Verification items for the finished model (mm, model axes). A direction names the side the tool comes from. Round coordinates to 2 decimals unless told otherwise and drop trailing zeros. Order: outer loops, then holes, each group sorted by start corner. A loop starts at its lowest first (then second) coordinate and runs counter-clockwise, first axis right, second up. Notation, with made-up numbers: (48.25, -22) -> (74.25, -22) arc R18 ccw to (74.25, 0) -> close; hole circle Ø4 at (51, 29.25). An arc over 180 degrees is marked (long way). Put each result on its own line as item: value.
from build123d import *

# Parameters (mm, degrees)
SQUARE_FLANGE_SKETCH_R           = 1
SQUARE_FLANGE_SKETCH_R_2         = 0.265
SQUARE_OUTLET_FLANGE_DEPTH       = 0.65
ROUND_FLANGE_HOLES_SKETCH_R      = 0.375
ROUND_FLANGE_HOLES_4X_0_75_DEPTH = 0.65
ROUND_FLANGE_HOLE_CHAMFERS_SIZE  = 0.0325
SQUARE_FLANGE_CHAMFERS_SIZE      = 0.0325
HOUSING_EDGE_CHAMFERS_SIZE       = 0.125


with BuildPart() as part:
    # Housing Profile Sketch → Housing Body Revolve (revolve)
    with BuildSketch(Plane.XY, mode=Mode.PRIVATE) as housing_body_revolve_sk:
        Polygon((0, 1), (0, 1.8125), (0.063, 1.8755), (0.063, 3), (0.65, 3), (0.65, 1.504103507), (1.375, 1.35), (2.125, 1.35), (2.125, 1.812), (2.188, 1.875), (2.188, 1), align=None)
    revolve(housing_body_revolve_sk.sketch.rotate(Axis((0, 0, 0), (1, 0, 0)), 90), axis=Axis((0, 0, 0), (1, 0, 0)))

    # Square Flange Sketch → Square Outlet Flange (add)
    with BuildSketch(Plane(origin=(2.188, 0, 0), x_dir=(0, 0, -1), z_dir=(1, 0, 0))):
        with BuildLine():
            Line((-1.594555277, 2.361757009), (-1.047699115, 2.375349419))
            ThreePointArc((-1.047699115, 2.375349419), (-0.801459389, 2.393837984), (-0.558303573, 2.436862146))
            ThreePointArc((-0.558303573, 2.436862146), (0.0283118, 2.499839683), (0.613350393, 2.423592642))
            ThreePointArc((0.613350393, 2.423592642), (0.974691231, 2.360294751), (1.341424141, 2.351306033))
            Line((1.341424141, 2.351306033), (1.535705916, 2.361018432))
            ThreePointArc((1.535705916, 2.361018432), (2.110295851, 2.15191191), (2.361757009, 1.594555277))
            Line((2.361757009, 1.594555277), (2.375349419, 1.047699115))
            ThreePointArc((2.375349419, 1.047699115), (2.393837984, 0.801459389), (2.436862146, 0.558303573))
            ThreePointArc((2.436862146, 0.558303573), (2.499839683, -0.0283118), (2.423592642, -0.613350393))
            ThreePointArc((2.423592642, -0.613350393), (2.360294751, -0.974691231), (2.351306033, -1.341424141))
            Line((2.351306033, -1.341424141), (2.361018432, -1.535705916))
            ThreePointArc((2.361018432, -1.535705916), (2.15191191, -2.110295851), (1.594555277, -2.361757009))
            Line((1.594555277, -2.361757009), (1.047699115, -2.375349419))
            ThreePointArc((1.047699115, -2.375349419), (0.801459389, -2.393837984), (0.558303573, -2.436862146))
            ThreePointArc((0.558303573, -2.436862146), (-0.0283118, -2.499839683), (-0.613350393, -2.423592642))
            ThreePointArc((-0.613350393, -2.423592642), (-0.974691231, -2.360294751), (-1.341424141, -2.351306033))
            Line((-1.341424141, -2.351306033), (-1.535705916, -2.361018432))
            ThreePointArc((-1.535705916, -2.361018432), (-2.110295851, -2.15191191), (-2.361757009, -1.594555277))
            Line((-2.361757009, -1.594555277), (-2.375349419, -1.047699115))
            ThreePointArc((-2.375349419, -1.047699115), (-2.393837984, -0.801459389), (-2.436862146, -0.558303573))
            ThreePointArc((-2.436862146, -0.558303573), (-2.499839683, 0.0283118), (-2.423592642, 0.613350393))
            ThreePointArc((-2.423592642, 0.613350393), (-2.360294751, 0.974691231), (-2.351306033, 1.341424141))
            Line((-2.351306033, 1.341424141), (-2.361018432, 1.535705916))
            ThreePointArc((-2.361018432, 1.535705916), (-2.15191191, 2.110295851), (-1.594555277, 2.361757009))
        make_face()
        with Locations(Location((0, 0, 0), (0, 0, 180))):
            Circle(SQUARE_FLANGE_SKETCH_R, mode=Mode.SUBTRACT)
        with Locations((-1.679378605, 1.679378605)):
            Circle(SQUARE_FLANGE_SKETCH_R_2, mode=Mode.SUBTRACT)
        with Locations((1.679378605, 1.679378605)):
            Circle(SQUARE_FLANGE_SKETCH_R_2, mode=Mode.SUBTRACT)
        with Locations((1.679378605, -1.679378605)):
            Circle(SQUARE_FLANGE_SKETCH_R_2, mode=Mode.SUBTRACT)
        with Locations((-1.679378605, -1.679378605)):
            Circle(SQUARE_FLANGE_SKETCH_R_2, mode=Mode.SUBTRACT)
    extrude(amount=SQUARE_OUTLET_FLANGE_DEPTH)

    # Round Flange Holes Sketch → Round Flange Holes 4xØ0.75 (cut)
    with BuildSketch(Plane.ZY.offset(-0.063)):
        with Locations((-1.575, 1.777638883)):
            Circle(ROUND_FLANGE_HOLES_SKETCH_R)
        with Locations((1.777638883, 1.575)):
            Circle(ROUND_FLANGE_HOLES_SKETCH_R)
        with Locations((1.575, -1.777638883)):
            Circle(ROUND_FLANGE_HOLES_SKETCH_R)
        with Locations((-1.777638883, -1.575)):
            Circle(ROUND_FLANGE_HOLES_SKETCH_R)
    extrude(amount=-ROUND_FLANGE_HOLES_4X_0_75_DEPTH, mode=Mode.SUBTRACT)

    # Round Flange Hole Chamfers
    round_flange_hole_chamfers_edges = [part.edges().sort_by_distance(p)[0] for p in [
        (0.65, -1.777638883, 1.2),
        (0.063, -1.777638883, 1.2),
        (0.65, 1.575, 1.402638883),
        (0.063, 1.575, 1.402638883),
        (0.65, 1.777638883, -1.95),
        (0.063, 1.777638883, -1.95),
        (0.65, -1.575, -2.152638883),
        (0.063, -1.575, -2.152638883),
    ]]
    chamfer(round_flange_hole_chamfers_edges, length=ROUND_FLANGE_HOLE_CHAMFERS_SIZE)

    # Square Flange Chamfers
    square_flange_chamfers_edges = [part.edges().sort_by_distance(p)[0] for p in [
        (2.188, 1.679378605, 1.944378605),
        (2.188, 1.679378605, -1.414378605),
        (2.188, -1.679378605, -1.414378605),
        (2.188, -1.679378605, 1.944378605),
        (2.838, 1.679378605, 1.944378605),
        (2.838, 1.679378605, -1.414378605),
        (2.838, -1.679378605, -1.414378605),
        (2.838, -1.679378605, 1.944378605),
    ]]
    chamfer(square_flange_chamfers_edges, length=SQUARE_FLANGE_CHAMFERS_SIZE)

    # Housing Edge Chamfers
    housing_edge_chamfers_edges = [part.edges().sort_by_distance(p)[0] for p in [
        (0, 0, -1),
        (2.838, 0, -1),
    ]]
    chamfer(housing_edge_chamfers_edges, length=HOUSING_EDGE_CHAMFERS_SIZE)


solid = part.part
Item 1: Gauge pin test, flat end, axial feed: pin 1 Ø1.5 at (x, z) = (1, -1) entering from -Y. Record the tip position at first contact, or that the pin passes through.
Check sheet entries:
pin 1: stops at y = -2.98
Item 2: Release check for a two-part mould opening along Z. For faces 1 (the cylindrical face through (0.36, -0.9, 2.86)), 2 (the flat face through (0, 1, 1)), 3 (the cylindrical face through (1, 1, 0)) record: +Z half, -Z half, draft (parallel to the pull), parting line (faces both ways), or undercut.
Check sheet entries:
face 1: parting line
face 2: draft
face 3: undercut
Item 3: Material ranges on L1, parallel to Y at x = 2.65, z = 0; L2, parallel to X at y = -0.2, z = 1.95, recorded low to high. Write a range as [from, to].
Check sheet entries:
L1: y = [-2.5, -1], [1, 2.5]
L2: x = [0.06, 0.65], [2.19, 2.84]
Item 4: Section check D-D on x = 0.9. Record the boundary of the cut face in (y, z), then the cut area to 3 significant figures.
Check sheet entries:
outline: circle Ø2.9 at (0, 0); hole circle Ø2 at (0, 0)
area: 3.47 mm^2
Item 5: Section check C-C on x = 2.3. State how many separate pieces and enclosed holes the cut face has, then the cut area to 3 significant figures.
Check sheet entries:
separate pieces: 1
enclosed holes: 5
area: 18.4 mm^2
Item 6: Tool access check on faces 4 (the flat face through (0.65, 1.29, 1.29)), 5 (the flat face through (2.838, 1, -1)), 6 (the flat face through (0.063, 2, -1)). Record the directions out of +Z, -Z, +X, -X, +Y, -Y that give a thin tool (end or side, any length) a straight path to the whole face; none if there is none.
Check sheet entries:
face 4: none
face 5: +Z, -Z, +X, +Y, -Y
face 6: -X
